```python
from build123d import *

# Parameters (mm, degrees)
SKETCH_1_W                   = 50
SKETCH_1_H                   = 50
EXTRUDE_1_DEPTH              = 5
SKETCH_2_R                   = 20
CUT_EXTRUDE_1_DEPTH          = 37.742346142
HOLE_WIZARD_M5_1_D           = 5.8
HOLE_WIZARD_M5_1_CBORE_D     = 10
HOLE_WIZARD_M5_1_CBORE_DEPTH = 5.4
CHAMFER_1_SIZE               = 2
SKETCH_7_R                   = 20
SKETCH_7_R_2                 = 12.5
EXTRUDE_2_DEPTH              = 2.2


with BuildPart() as part:
    # 草图1 → 凸台-拉伸1 (new, symmetric)
    with BuildSketch(Plane.XY):
        Rectangle(SKETCH_1_W, SKETCH_1_H)
    extrude(amount=EXTRUDE_1_DEPTH, both=True)

    # 草图2 → 切除-拉伸1 (cut, through all)
    with BuildSketch(Plane.XY.offset(5)):
        Circle(SKETCH_2_R)
    extrude(amount=-CUT_EXTRUDE_1_DEPTH, mode=Mode.SUBTRACT)

    # M5 六角凹头螺钉的柱形沉头孔1 (through all)
    with Locations(Plane.XY.offset(5)):
        with Locations((-19, 19), (19, 19), (-19, -19), (19, -19)):
            CounterBoreHole(HOLE_WIZARD_M5_1_D / 2, HOLE_WIZARD_M5_1_CBORE_D / 2, HOLE_WIZARD_M5_1_CBORE_DEPTH)

    # 倒角1
    chamfer_1_edges = [part.edges().sort_by_distance(p)[0] for p in [
        (25, -25, 0),
        (-25, -25, 0),
        (-25, 25, 0),
        (25, 25, 0),
    ]]
    chamfer(chamfer_1_edges, length=CHAMFER_1_SIZE)

    # 草图7 → 凸台-拉伸2 (add)
    with BuildSketch(Plane.XY.offset(5)):
        Circle(SKETCH_7_R)
        Circle(SKETCH_7_R_2, mode=Mode.SUBTRACT)
    extrude(amount=-EXTRUDE_2_DEPTH)


solid = part.part
```
Part model, mm, in its own coordinate system. A direction names the side the tool comes from. Coordinates: 2 decimals unless noted, no trailing zeros. Order: outer loops, then holes, each group sorted by start corner. A loop starts at its lowest first (then second) coordinate and runs counter-clockwise, first axis right, second up. Notation, with made-up numbers: (4, 23.5) - (46, 23.5) arc R21 ccw to (46, 50.5) - close; hole circle Ø9 at (7, -8.75). An arc over 180 degrees is marked (long way). Return JSON: item names as keys, results as strings. Group by question number.
Item 1: Drill centre lines: probe 1 along Y at (x, z) = (0.5, 0.75); probe 2 along X at (y, z) = (-16.5, -2.75); probe 3 along X at (y, z) = (-20, 4). Where is each one in solid material? Low to high. Write a range as from..to.
Item 2: Pin check, flat tips, straight feed: pin 1 (9 mm diameter, centred on x = -19, y = -19, fed in from +Z); pin 2 (5 mm diameter, centred on x = 7, y = -14.5, fed in from -Z). Stop position of each tip, or through.
Item 3: Cut at B-B (x = 0). List the corners of the cut face in (y, z), plus the area to 3 significant figures.
Item 4: Which spindle directions (+Z, -Z, +X, -X, +Y, -Y) get a long thin tool onto all of the face, cutting with end or side? Do faces 5 (the face through (-25, 0, 0)), 6 (the face through (17.92, 14.12, 2.34)), 7 (the face through (9, 9, 2.8)). Say none if no direction does.
Item 5: Cut at D-D (x = 19). List the corners of the cut face in (y, z) (3 decimals).
Item 6: Cut at A-A (z = 2). List the corners of the cut face in (x, y), plus the area to 3 significant figures.
Item 7: Pull direction X, two halves, no side cores. Call faces 1 (the face through (25, 0, 0)), 2 (the face through (21.2, 16.8, -0.4)), 3 (the face through (-24, -24, 0)), 4 (the face through (-16.8, -21.2, -0.4)): pulls with the +X half, pulls with the -X half, needs draft (parallel to the pull), parting line crosses it, or undercut.
Check values:
{
 "1": {"probe 1": "y = -25..-19.99, 19.99..25", "probe 2": "x = -25..-20.47, -17.53..-11.3, 11.3..17.53, 20.47..25", "probe 3": "x = -25..-23.9, -14.1..14.1, 23.9..25"},
 "2": {"pin 1": "stops at z = -0.4", "pin 2": "stops at z = 2.8"},
 "3": {"outline": "(-25, -5) - (-20, -5) - (-20, 2.8) - (-12.5, 2.8) - (-12.5, 5) - (-25, 5) - close; (12.5, 2.8) - (20, 2.8) - (20, -5) - (25, -5) - (25, 5) - (12.5, 5) - close", "area": "133 mm2"},
 "4": {"face 5": "+Z, -Z, -X, +Y, -Y", "face 6": "+Z", "face 7": "-Z"},
 "5": {"outline": "(-25, -5) - (-21.9, -5) - (-21.9, -0.4) - (-24, -0.4) - (-24, 5) - (-25, 5) - close; (-16.1, -5) - (-6.245, -5) - (-6.245, 2.8) - (6.245, 2.8) - (6.245, -5) - (16.1, -5) - (16.1, -0.4) - (14, -0.4) - (14, 5) - (-14, 5) - (-14, -0.4) - (-16.1, -0.4) - close; (21.9, -5) - (25, -5) - (25, 5) - (24, 5) - (24, -0.4) - (21.9, -0.4) - close"},
 "6": {"outline": "(-25, -23) - (-23, -25) - (23, -25) - (25, -23) - (25, 23) - (23, 25) - (-23, 25) - (-25, 23) - close; hole circle Ø10 at (-19, -19); hole circle Ø10 at (-19, 19); hole circle Ø40 at (0, 0); hole circle Ø10 at (19, -19); hole circle Ø10 at (19, 19)", "area": "921 mm2"},
 "7": {"face 1": "pulls with the +X half", "face 2": "undercut", "face 3": "pulls with the -X half", "face 4": "undercut"}
}
